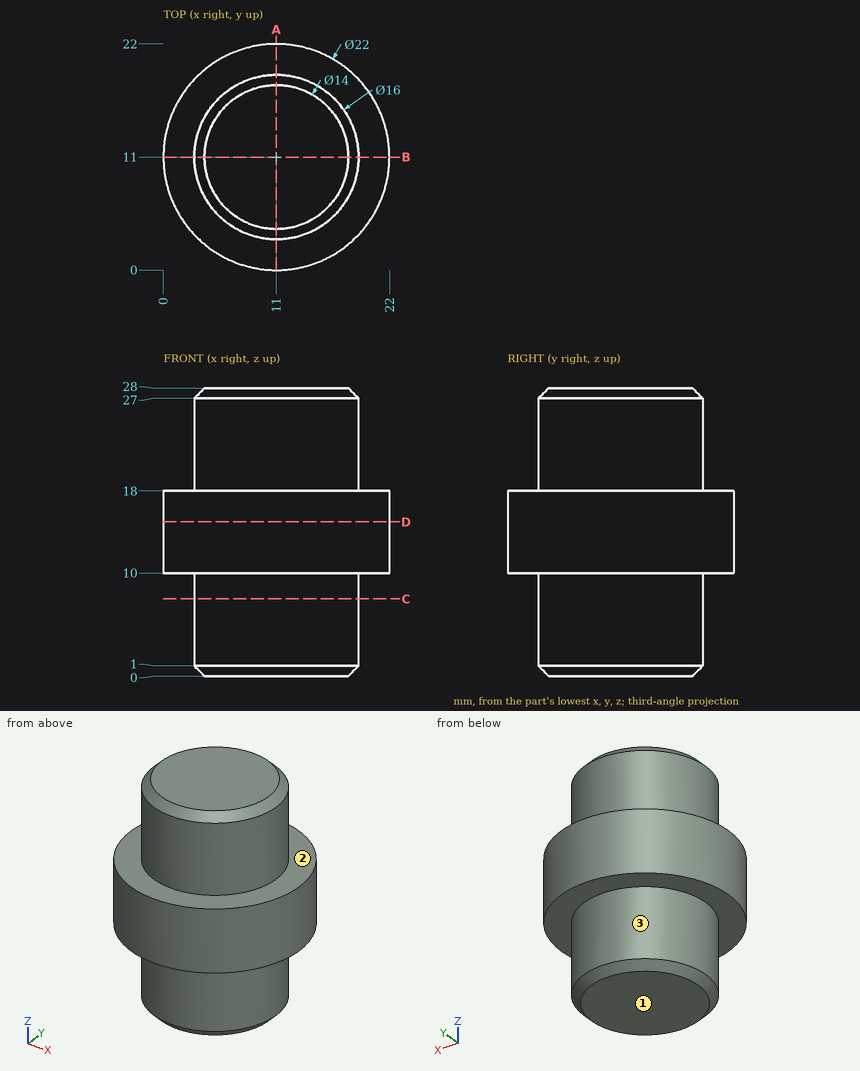
Part print with two shaded views. Sizes in mm from the minimum x, y, z corner. A direction names the side the tool comes from. Give positions to 0.01 mm unless a question says otherwise; leave off trailing zeros. Write each loop counter-clockwise with the first axis right and the second up, starting at its lowest first coordinate (ties: lowest second). Pieces come first, ordered by that corner, then holes.
1) Probe L1, parallel to Y at x = 10.75, z = 24.5; L2, parallel to Z at x = 15.5, y = 20; L3, parallel to X at y = 8.5, z = 19. List the from-to ranges inside material, lowest first.
Resolved:
L1: y = 3 to 19
L2: z = 10 to 18
L3: x = 3.4 to 18.6
2) Cut at D-D on z = 15. Write the cut outline in (x, y).
Resolved:
outline: circle Ø22 at (11, 11)
3) Cut at C-C on z = 7.5. Write the cut outline in (x, y), then the cut area to 3 significant figures.
Resolved:
outline: circle Ø16 at (11, 11)
area: 201 mm2
4) Pin check, flat tips, straight feed: pin 1 (4 mm diameter, centred on x = 3.5, z = 7.5, fed in from +Y); pin 2 (5 mm diameter, centred on x = 15, z = 14.5, fed in from -Y); pin 3 (1 mm diameter, centred on y = 10, z = 20.5, fed in from -X). Stop position of each tip, or through.
Resolved:
pin 1: stops at y = 16.81
pin 2: stops at y = 0.1
pin 3: stops at x = 3.02
5) Cut at A-A on x = 11. Write the cut outline in (y, z), then the cut area to 3 significant figures.
Resolved:
outline: (0, 10) - (3, 10) - (3, 1) - (4, 0) - (18, 0) - (19, 1) - (19, 10) - (22, 10) - (22, 18) - (19, 18) - (19, 27) - (18, 28) - (4, 28) - (3, 27) - (3, 18) - (0, 18) - close
area: 494 mm2
6) Which spindle directions (+Z, -Z, +X, -X, +Y, -Y) get a long thin tool onto all of the face, cutting with end or side? Do the marked faces 1, 2 and 3. Say none if no direction does.
Resolved:
face 1: -Z, +X, -X, +Y, -Y
face 2: +Z
face 3: -Z
